Check sheet for the modelled part. Datum: model origin and axes. Units: mm. Face numbers are marked on the shaded views. A direction names the side the tool comes from. Round coordinates to 2 decimals unless told otherwise and drop trailing zeros. Loops run counter-clockwise (first coordinate to the right, second up) from the corner with the lowest first, then second, coordinate; pieces in that order, holes last. Notation, with made-up numbers: (-11, 42.25) -> (31, 42.25) arc R16 cw to (31, 70.25) -> close; hole circle Ø5 at (75.5, -2). An arc over 180 degrees is marked (long way). One line per question, with ' | ' between items.
```python
from build123d import *

# Parameters (mm, degrees)
BASE_BLOCK_SKETCH_W        = 108
BASE_BLOCK_SKETCH_H        = 50
BASE_BLOCK_108X50X28_DEPTH = 14
END_CHAMFER_11X45DEG_SIZE  = 11
THROUGH_BORE_SKETCH_R      = 14
THROUGH_BORE_DEPTH         = 28
SLOT_RECESS_6_DEEP_DEPTH   = 6
ARC_RECESS_6_DEEP_DEPTH    = 6
ARC_HOLES_SKETCH_R         = 5
HOLES_2XD10_ON_R100_DEPTH  = 22
GROOVE_6_DEEP_DEPTH        = 6


with BuildPart() as part:
    # Base Block Sketch → Base Block 108x50x28 (new, symmetric)
    with BuildSketch(Plane(origin=(0, 0, 0), x_dir=(1, 0, 0), z_dir=(0, 1, 0))):
        Rectangle(BASE_BLOCK_SKETCH_W, BASE_BLOCK_SKETCH_H)
    extrude(amount=BASE_BLOCK_108X50X28_DEPTH, both=True)

    # End Chamfer 11x45deg
    end_chamfer_11x45deg_edges = [part.edges().sort_by_distance(p)[0] for p in [
        (54, 0, 25),
        (54, 0, -25),
    ]]
    chamfer(end_chamfer_11x45deg_edges, length=END_CHAMFER_11X45DEG_SIZE)

    # Through Bore Sketch → Through Bore (cut)
    with BuildSketch(Plane(origin=(0, 14, 0), x_dir=(1, 0, 0), z_dir=(0, 1, 0))):
        with Locations(Location((14, 0, 0), (0, 0, 270))):
            Circle(THROUGH_BORE_SKETCH_R)
    extrude(amount=-THROUGH_BORE_DEPTH, mode=Mode.SUBTRACT)

    # Slot Recess Sketch → Slot Recess 6 Deep (cut)
    with BuildSketch(Plane(origin=(0, 14, 0), x_dir=(1, 0, 0), z_dir=(0, 1, 0))):
        Polygon((1, 25), (1, -25), (43, -25), (54, -14), (54, 14), (43, 25), align=None)
    extrude(amount=-SLOT_RECESS_6_DEEP_DEPTH, mode=Mode.SUBTRACT)

    # Arc Recess Sketch → Arc Recess 6 Deep (cut)
    with BuildSketch(Plane(origin=(0, 14, 0), x_dir=(1, 0, 0), z_dir=(0, 1, 0))):
        with BuildLine():
            Line((-40.543560573, -25), (-17.224989992, -25))
            ThreePointArc((-17.224989992, -25), (-26, 0), (-17.224989992, 25))
            Line((-17.224989992, 25), (-40.543560573, 25))
            ThreePointArc((-40.543560573, 25), (-46, 0), (-40.543560573, -25))
        make_face()
    extrude(amount=-ARC_RECESS_6_DEEP_DEPTH, mode=Mode.SUBTRACT)

    # Arc Holes Sketch → Holes 2xD10 on R100 (cut)
    with BuildSketch(Plane(origin=(0, 8, 0), x_dir=(1, 0, 0), z_dir=(0, 1, 0))):
        with Locations(Location((-33.552825815, 15.450849719, 0), (0, 0, 270))):
            Circle(ARC_HOLES_SKETCH_R)
        with Locations(Location((-33.552825815, -15.450849719, 0), (0, 0, 270))):
            Circle(ARC_HOLES_SKETCH_R)
    extrude(amount=-HOLES_2XD10_ON_R100_DEPTH, mode=Mode.SUBTRACT)

    # Groove Sketch → Groove 6 Deep (cut)
    with BuildSketch(Plane(origin=(0, 8, 0), x_dir=(1, 0, 0), z_dir=(0, 1, 0))):
        with BuildLine():
            Line((25.904726429, 7.367325747), (54, 7.367325747))
            Line((54, 7.367325747), (54, -7.367325747))
            Line((54, -7.367325747), (25.904726429, -7.367325747))
            ThreePointArc((25.904726429, -7.367325747), (28, 0), (25.904726429, 7.367325747))
        make_face()
    extrude(amount=-GROOVE_6_DEEP_DEPTH, mode=Mode.SUBTRACT)


solid = part.part
```
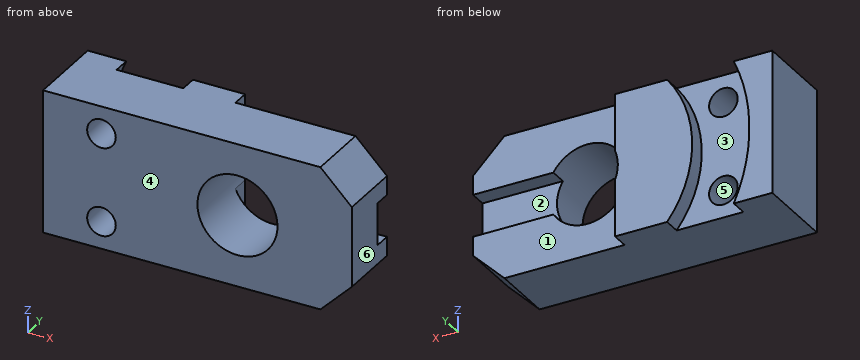
(1) Sectioned sample at D-D, the plane x = -35. Record the cut outline in (y, z), and give its area (3 significant figures).
Answer:
outline: (-14, -25) -> (8, -25) -> (8, -20.24) -> (-14, -20.24) -> close; (-14, -10.66) -> (8, -10.66) -> (8, 10.66) -> (-14, 10.66) -> close; (-14, 20.24) -> (8, 20.24) -> (8, 25) -> (-14, 25) -> close | area: 679 mm2
(2) Set-up check for the marked faces 1, 2 and 3: record each of +Z, -Z, +X, -X, +Y, -Y from which the full face is reachable in a straight line by a thin tool's end or side.
Answer:
face 1: +Z, -Z, +X, +Y | face 2: +X, +Y | face 3: +Y
(3) Sectioned sample at A-A, the plane x = 14. Record the cut outline in (y, z), and give its area (3 significant figures).
Answer:
outline: (-14, -25) -> (8, -25) -> (8, -14) -> (-14, -14) -> close; (-14, 14) -> (8, 14) -> (8, 25) -> (-14, 25) -> close | area: 484 mm2
(4) Mould release check, pull along X, two halves, no side actions. Record for the marked faces 4, 5 and 6: +X half, -X half, draft (parallel to the pull), parting line (faces both ways), or undercut.
Answer:
face 4: draft | face 5: undercut | face 6: +X half
(5) Go/stop test with flat-tipped pins: pin 1 (6.5 mm diameter, centred on y = 11.5, z = 16, fed in from +X); pin 2 (22 mm diameter, centred on x = 24.5, z = 13.5, fed in from +Y); pin 3 (3 mm diameter, centred on x = 31.5, z = 0.5, fed in from +Y). Record where each tip stops, or that it passes through.
Answer:
pin 1: stops at x = 1 | pin 2: stops at y = 8 | pin 3: stops at y = 2
(6) Scan lines: probe 1 along Z at (x, y) = (14, -7.5); probe 2 along X at (y, z) = (7.75, 12.5); probe 3 along Y at (x, z) = (-31.5, -3). Record each from-to range of solid material in increasing order.
Answer:
probe 1: z = -25 to -14, 14 to 25 | probe 2: x = -54 to -37.59, -29.52 to 7.7, 20.3 to 54 | probe 3: y = -14 to 8
(7) Sectioned sample at C-C, the plane z = 0. Record the cut outline in (x, y).
Answer:
outline: (-54, -14) -> (0, -14) -> (0, 14) -> (-26, 14) -> (-26, 8) -> (-46, 8) -> (-46, 14) -> (-54, 14) -> close; (28, -14) -> (54, -14) -> (54, 2) -> (28, 2) -> close
(8) Sectioned sample at B-B, the plane y = 11.5. Record the cut outline in (x, z).
Answer:
outline: (-54, -25) -> (-40.54, -25) arc R60 cw to (-40.54, 25) -> (-54, 25) -> close; (-17.22, -25) -> (1, -25) -> (1, -5.2) arc R14 cw to (1, 5.2) -> (1, 25) -> (-17.22, 25) arc R40 ccw to start
